```python
from build123d import *

# Parameters (mm, degrees)
SKETCH1_W           = 30
SKETCH1_H           = 178
BOSS_EXTRUDE1_DEPTH = 5
SKETCH3_W           = 26
SKETCH3_H           = 210
CUT_EXTRUDE1_DEPTH  = 3
SKETCH4_W           = 26
SKETCH4_H           = 10
BOSS_EXTRUDE2_DEPTH = 3
CUT_EXTRUDE3_DEPTH  = 5
BOSS_EXTRUDE3_START = 3
BOSS_EXTRUDE3_DEPTH = 3


with BuildPart() as part:
    # Sketch1 → Boss-Extrude1 (new body)
    with BuildSketch(Plane.XY):
        with Locations((15, 89)):
            Rectangle(SKETCH1_W, SKETCH1_H)
    extrude(amount=BOSS_EXTRUDE1_DEPTH)

    # Sketch3 → Cut-Extrude1 (cut)
    with BuildSketch(Plane.XY.offset(5)):
        with Locations((15, 71)):
            Rectangle(SKETCH3_W, SKETCH3_H)
    extrude(amount=-CUT_EXTRUDE1_DEPTH, mode=Mode.SUBTRACT)

    # Sketch4 → Boss-Extrude2 (add)
    with BuildSketch(Plane.XY.offset(2)):
        with Locations((15, 23)):
            Rectangle(SKETCH4_W, SKETCH4_H)
    extrude(amount=BOSS_EXTRUDE2_DEPTH)

    # Sketch5 → Cut-Extrude3 (cut, symmetric)
    with BuildSketch(Plane.XY.offset(2)):
        with BuildLine():
            Line((0, 0), (30, 0))
            ThreePointArc((30, 0), (15, 15), (0, 0))
        make_face()
    extrude(amount=CUT_EXTRUDE3_DEPTH, both=True, mode=Mode.SUBTRACT)

    # Sketch6 → Boss-Extrude3 (add)
    with BuildSketch(Plane.XY.offset(2).offset(BOSS_EXTRUDE3_START)):
        with BuildLine():
            Line((28, 7.483314774), (28, 18))
            Line((28, 18), (2, 18))
            Line((2, 18), (2, 7.483314774))
            ThreePointArc((2, 7.483314774), (15, 15), (28, 7.483314774))
        make_face()
    extrude(amount=-BOSS_EXTRUDE3_DEPTH)


solid = part.part
```
The model under review builds one solid part; all positions refer to its coordinate system, in mm. A direction names the side the tool comes from. Give positions to 0.01 mm unless a question says otherwise; leave off trailing zeros. Write each loop counter-clockwise with the first axis right and the second up, starting at its lowest first coordinate (ties: lowest second). Pieces come first, ordered by that corner, then holes.
(1) To check wall thickness, follow L1, parallel to X at y = 170, z = 4.65; L2, parallel to Y at x = 15, z = 2.7; L3, parallel to Z at x = 12, y = 34. State the ranges of each line that lie inside material, in increasing order.
(2) For P1, Ø2.5, axis at x = 19.5, z = 4, coming from the -Y side; P2, Ø13, axis at x = 10.5, y = 108, coming from the +Z side, all flat-tipped, find the tip position at first contact; note any pin that passes through.
(3) Tool access review of faces 1 (the flat face through (28, 101, 4)), 2 (the flat face through (15, 90, 0)): name each direction out of +Z, -Z, +X, -X, +Y, -Y from which nothing blocks a thin tool from reaching the whole face with its end or side.
(4) Consider section B-B, the plane z = 3.3. Give the boundary of the cut face in (x, y), and give its area (3 significant figures).
(5) Consider section C-C, the plane x = 15. Give the boundary of the cut face in (y, z), and give its area (3 significant figures).
(6) Consider section A-A, the plane y = 134. Give the boundary of the cut face in (x, z), and give its area (3 significant figures).
Returned:
1. L1: x = 0 to 2, 28 to 30
1. L2: y = 15 to 28, 176 to 178
1. L3: z = 0 to 2
2. P1: stops at y = 13.85
2. P2: stops at z = 2
3. face 1: +Z
3. face 2: -Z, +X, -X, +Y, -Y
4. outline: (0, 0) arc R15 cw to (30, 0) - (30, 178) - (0, 178) - close; hole (2, 28) - (28, 28) - (28, 176) - (2, 176) - close
4. area: 1,140 mm2
5. outline: (15, 0) - (178, 0) - (178, 5) - (176, 5) - (176, 2) - (28, 2) - (28, 5) - (15, 5) - close
5. area: 371 mm2
6. outline: (0, 0) - (30, 0) - (30, 5) - (28, 5) - (28, 2) - (2, 2) - (2, 5) - (0, 5) - close
6. area: 72.0 mm2
